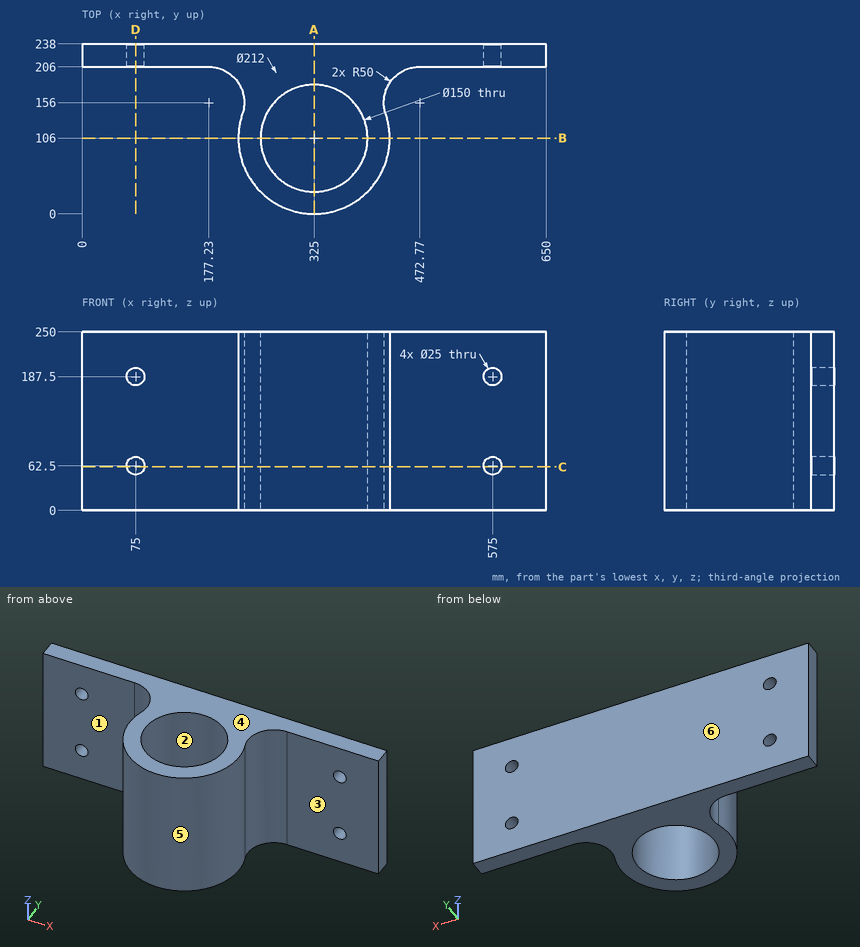
Geometry: see drawing. Coordinates: mm, zero at the bounding-box minimum. A direction names the side the tool comes from. Coordinates: 2 decimals unless noted, no trailing zeros. Loops run counter-clockwise (first coordinate to the right, second up) from the corner with the lowest first, then second, coordinate; pieces in that order, holes last. Notation, with made-up numbers: (10.5, 73.25) -> (47.5, 73.25) arc R16 ccw to (47.5, 80.25) -> close; hole circle Ø3 at (46, 56.25). An arc over 180 degrees is marked (long way). Write item = value, one per line. Start each with the question number.
Item 1: First-contact query: P1, Ø4, axis at y = 131, z = 219.5, coming from the -X side; P2, Ø3, axis at x = 512, z = 54.5, coming from the -Y side; P3, Ø6, axis at y = 189.5, z = 134.5, coming from the +X side. Flat tips, straight axial feed; report the tip coordinate or a pass-through.
Item 2: Cut plane A-A, the plane x = 325. Return loops of the section in (y, z), plus the area to 3 significant figures.
Item 3: Cut plane B-B, the plane y = 106. Return loops of the section in (x, z).
Item 4: Cut plane D-D, the plane x = 75. Return loops of the section in (y, z), plus the area to 3 significant figures.
Item 5: Cut plane C-C, the plane z = 61. Return loops of the section in (x, y).
Item 6: Reachability of the marked faces 1, 2 and 3 from +Z, -Z, +X, -X, +Y, -Y: full face, straight path, thin tool, end or side. Return the list, or none.
Item 7: Material intervals for line 1 (X direction, y = 221.5, z = 62.5); line 2 (X direction, y = 104.5, z = 40) (1 decimal); line 3 (Y direction, x = 325, z = 165), sorted ascending.
Item 8: Mould query, pull axis Y, two halves, no side actions, for the marked faces 4, 5 and 6. Classes: pulls with the +Y half, pulls with the -Y half, needs draft (parallel to the pull), parting line crosses it, or undercut.
Ans:
q1.P1 = 221.53
q1.P2 = 206
q1.P3 = 438.6
q2.outline = (0, 0) -> (31, 0) -> (31, 250) -> (0, 250) -> close; (181, 0) -> (238, 0) -> (238, 250) -> (181, 250) -> close
q2.area = 22,000 mm²
q3.outline = (219, 0) -> (250, 0) -> (250, 250) -> (219, 250) -> close; (400, 0) -> (431, 0) -> (431, 250) -> (400, 250) -> close
q4.outline = (206, 0) -> (238, 0) -> (238, 50) -> (206, 50) -> close; (206, 75) -> (238, 75) -> (238, 175) -> (206, 175) -> close; (206, 200) -> (238, 200) -> (238, 250) -> (206, 250) -> close
q4.area = 6,400 mm²
q5.outline = (0, 206) -> (62.59, 206) -> (62.59, 238) -> (0, 238) -> close; (87.41, 206) -> (177.23, 206) arc R50 cw to (224.59, 139.97) arc R106 ccw (long way) to (425.41, 139.97) arc R50 cw to (472.77, 206) -> (562.59, 206) -> (562.59, 238) -> (87.41, 238) -> close; (587.41, 206) -> (650, 206) -> (650, 238) -> (587.41, 238) -> close; hole circle Ø150 at (325, 106)
q6.face_1 = +Z, -Z, -X, -Y
q6.face_2 = +Z, -Z
q6.face_3 = +Z, -Z, +X, -Y
q7.line_1 = 0 to 62.5, 87.5 to 562.5, 587.5 to 650
q7.line_2 = 219 to 250, 400 to 431
q7.line_3 = 0 to 31, 181 to 238
q8.face_4 = needs draft
q8.face_5 = undercut
q8.face_6 = pulls with the +Y half
